```python
from build123d import *

# Parameters (mm, degrees)
SKETCH_1_W                = 57
SKETCH_1_H                = 55
EXTRUDE_1_DEPTH           = 10
SKETCH_2_W                = 16
SKETCH_2_H                = 35
CUT_EXTRUDE_1_DEPTH       = 41.847276531
HOLE_WIZARD_1_D           = 4.8
HOLE_WIZARD_1_CBORE_D     = 8
HOLE_WIZARD_1_CBORE_DEPTH = 6.6
HOLE_WIZARD_M3_1_D        = 2.5
FILLET_1_R                = 5
SKETCH_8_W                = 10
SKETCH_8_H                = 55
EXTRUDE_2_DEPTH           = 15
HOLE_WIZARD_2_D           = 5.5
HOLE_WIZARD_2_CBORE_D     = 10
HOLE_WIZARD_2_CBORE_DEPTH = 5.7
SKETCH_11_W               = 25
SKETCH_11_H               = 2
CUT_EXTRUDE_2_DEPTH       = 2
CHAMFER_3_SIZE            = 2
CHAMFER_4_SIZE            = 1


with BuildPart() as part:
    # 草图1 → 凸台-拉伸1 (new body)
    with BuildSketch(Plane.XY):
        Rectangle(SKETCH_1_W, SKETCH_1_H)
    extrude(amount=EXTRUDE_1_DEPTH)

    # 草图2 → 切除-拉伸1 (cut, through all)
    with BuildSketch(Plane.XY.offset(10)):
        with Locations((-8.5, 0)):
            Rectangle(SKETCH_2_W, SKETCH_2_H)
    extrude(amount=-CUT_EXTRUDE_1_DEPTH, mode=Mode.SUBTRACT)

    # 打孔尺寸(%根据)内六角圆柱头螺钉的类型1 (through all)
    with Locations(Plane.XY.offset(10)):
        with Locations((-21, 20), (4, 20), (-21, -20), (4, -20)):
            CounterBoreHole(HOLE_WIZARD_1_D / 2, HOLE_WIZARD_1_CBORE_D / 2, HOLE_WIZARD_1_CBORE_DEPTH)

    # M3 螺纹孔1 (through all)
    with Locations(Plane.XY.offset(10)):
        with Locations((-21, 10), (-21, -10), (4, 10), (4, -10)):
            Hole(HOLE_WIZARD_M3_1_D / 2)

    # 圆角1
    fillet_1_edges = [part.edges().sort_by_distance(p)[0] for p in [
        (-16.5, -17.5, 5),
        (-16.5, 17.5, 5),
        (-0.5, 17.5, 5),
        (-0.5, -17.5, 5),
    ]]
    fillet(fillet_1_edges, radius=FILLET_1_R)

    # 草图8 → 凸台-拉伸2 (add)
    with BuildSketch(Plane.XY.offset(10)):
        with Locations((23.5, 0)):
            Rectangle(SKETCH_8_W, SKETCH_8_H)
    extrude(amount=EXTRUDE_2_DEPTH)

    # 打孔尺寸(%根据)内六角圆柱头螺钉的类型2 (through all)
    with Locations(Plane.ZY.offset(-18.5)):
        with Locations((17.5, 20), (17.5, 0), (17.5, -20)):
            CounterBoreHole(HOLE_WIZARD_2_D / 2, HOLE_WIZARD_2_CBORE_D / 2, HOLE_WIZARD_2_CBORE_DEPTH)

    # 草图11 → 切除-拉伸2 (cut)
    with BuildSketch(Plane(origin=(28.5, 0, 0), x_dir=(0, 0, -1), z_dir=(1, 0, 0))):
        with Locations((-12.5, 26.5)):
            Rectangle(SKETCH_11_W, SKETCH_11_H)
        with Locations((-12.5, -26.5)):
            Rectangle(SKETCH_11_W, SKETCH_11_H)
    extrude(amount=-CUT_EXTRUDE_2_DEPTH, mode=Mode.SUBTRACT)

    # 倒角3
    chamfer_3_edges = [part.edges().sort_by_distance(p)[0] for p in [
        (-28.5, -27.5, 5),
        (-28.5, 27.5, 5),
    ]]
    chamfer(chamfer_3_edges, length=CHAMFER_3_SIZE)

    # 倒角4
    chamfer_4_edges = [part.edges().sort_by_distance(p)[0] for p in [
        (22.5, -27.5, 25),
        (22.5, 27.5, 25),
    ]]
    chamfer(chamfer_4_edges, length=CHAMFER_4_SIZE)


solid = part.part
```
Model file for the job. Use its own axes, mm. A direction names the side the tool comes from. Give positions to 0.01 mm unless a question says otherwise; leave off trailing zeros. Loops run counter-clockwise (first coordinate to the right, second up) from the corner with the lowest first, then second, coordinate; pieces in that order, holes last. Notation, with made-up numbers: (-23.75, -24) - (-15.75, -24) arc R22 ccw to (-15.75, 8) - close; hole circle Ø4 at (72.25, 79.25). An arc over 180 degrees is marked (long way). One line per item, written item: value. Start each with the question number.
1. Pin check, flat tips, straight feed: pin 1 (1.6 mm diameter, centred on x = 28, z = 14, fed in from +Y); pin 2 (9 mm diameter, centred on x = 4, y = 20.5, fed in from +Z); pin 3 (6 mm diameter, centred on y = 20.5, z = 20, fed in from -X). Stop position of each tip, or through.
2. Slice it at B-B (y = -10). List the corners of the cut face in (x, z), plus the area to 3 significant figures.
3. Pull direction Z, two halves, no side cores. Call faces 5 (the cylindrical face through (-20.48, 17.657, 1.676)), 6 (the cylindrical face through (21.31, 0.22, 12.505)), 7 (the flat face through (-19, 18, 3.4)): pulls with the +Z half, pulls with the -Z half, needs draft (parallel to the pull), parting line crosses it, or undercut.
4. Slice it at A-A (x = -8.5). List the corners of the cut face in (y, z).
5. Slice it at C-C (x = 21). List the corners of the cut face in (y, z).
6. Slice it at D-D (y = 0). List the corners of the cut face in (x, z), plus the area to 3 significant figures.
7. Which spindle directions (+Z, -Z, +X, -X, +Y, -Y) get a long thin tool onto all of the face, cutting with end or side? Do faces 1 (the cylindrical face through (-23.95, -17.3, 6.75)), 2 (the flat face through (28, 25.5, 13)), 3 (the flat face through (-9, 17.5, 5)), 4 (the flat face through (18.5, 0, 12)). Say none if no direction does.
8. Probe L1, parallel to Y at x = 27.3, z = 17.5; L2, parallel to Y at x = -9, z = 8.5; L3, parallel to Z at x = 7, y = 21. List the from-to ranges inside material, lowest first. Write a range as from..to.
Solution:
1. pin 1: stops at y = 25.5
1. pin 2: stops at z = 10
1. pin 3: stops at x = 18.5
2. outline: (-28.5, 0) - (-22.25, 0) - (-22.25, 10) - (-28.5, 10) - close; (-19.75, 0) - (-16.5, 0) - (-16.5, 10) - (-19.75, 10) - close; (-0.5, 0) - (2.75, 0) - (2.75, 10) - (-0.5, 10) - close; (5.25, 0) - (28.5, 0) - (28.5, 25) - (18.5, 25) - (18.5, 10) - (5.25, 10) - close
2. area: 510 mm^2
3. face 5: needs draft
3. face 6: undercut
3. face 7: pulls with the +Z half
4. outline: (-27.5, 0) - (-17.5, 0) - (-17.5, 10) - (-27.5, 10) - close; (17.5, 0) - (27.5, 0) - (27.5, 10) - (17.5, 10) - close
5. outline: (-27.5, 0) - (27.5, 0) - (27.5, 24) - (26.5, 25) - (-26.5, 25) - (-27.5, 24) - close; hole circle Ø10 at (-20, 17.5); hole circle Ø10 at (0, 17.5); hole circle Ø10 at (20, 17.5)
6. outline: (-28.5, 0) - (-16.5, 0) - (-16.5, 10) - (-28.5, 10) - close; (-0.5, 0) - (28.5, 0) - (28.5, 14.75) - (24.2, 14.75) - (24.2, 12.5) - (18.5, 12.5) - (18.5, 10) - (-0.5, 10) - close; (18.5, 22.5) - (24.2, 22.5) - (24.2, 20.25) - (28.5, 20.25) - (28.5, 25) - (18.5, 25) - close
6. area: 479 mm^2
7. face 1: +Z
7. face 2: +Z, -Z, +X, +Y
7. face 3: +Z, -Z
7. face 4: +Z, -X, +Y, -Y
8. L1: y = -25.5..-22.75, -17.25..-2.75, 2.75..17.25, 22.75..25.5
8. L2: y = -27.5..-17.5, 17.5..27.5
8. L3: z = 0..3.4
